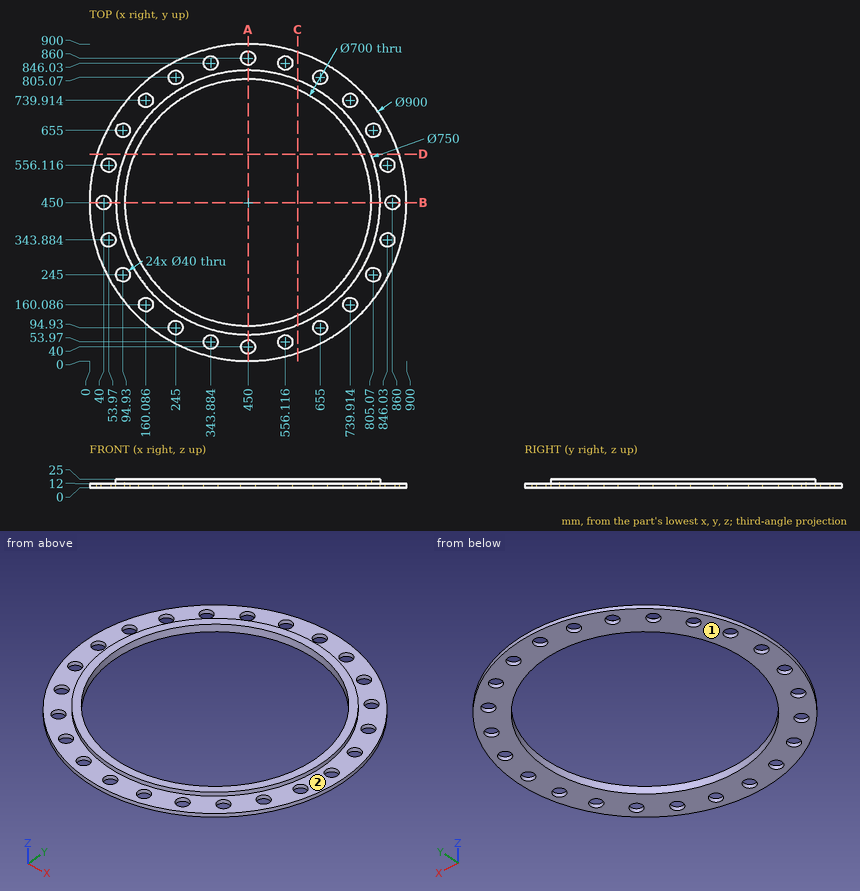
For this review, use the dimensioned drawing (mm, ordinates from the lowest corner) and the shaded views. A direction names the side the tool comes from. Coordinates: 2 decimals unless noted, no trailing zeros. Loops run counter-clockwise (first coordinate to the right, second up) from the corner with the lowest first, then second, coordinate; pieces in that order, holes last. Notation, with made-up numbers: (60, 67.5) -> (105, 67.5) arc R18 cw to (105, 101.5) -> close; hole circle Ø11 at (89, 46). An arc over 180 degrees is marked (long way). Use a Markdown table: item, result. Add a question column.
1. To check wall thickness, follow line 1 (X direction, y = 847, z = 7.25) (1 decimal); line 2 (X direction, y = 860, z = 3) (1 decimal); line 3 (Z direction, x = 248.5, y = 848). State the ranges of each line that lie inside material, in increasing order.
2. Add section A-A on x = 450. Write out the cut boundary in (y, z), plus the area to 3 significant figures.
3. Clearance check with flat-ended pins moving along their axes: pin 1 Ø10 at (y, z) = (162, 11.5) entering from -X; pin 2 Ø24 at (x, y) = (94.93, 245) entering from +Z; pin 3 Ø2 at (x, z) = (487.5, 3.5) entering from -Y; pin 4 Ø1 at (y, z) = (552.5, 6.5) entering from +X. State where each tip first meets the part, or that it passes through.
4. Machinability: for the marked faces 1 and 2, which of the approach directions +Z, -Z, +X, -X, +Y, -Y give a long, thin tool a straight path to every point of the face, cutting with its end or side? Answer none if there is none.
5. Add section C-C on x = 591. Write out the cut boundary in (y, z).
6. Add section D-D on y = 587.5. Write out the cut boundary in (x, z), plus the area to 3 significant figures.
Returned:
| question | item | result |
|---|---|---|
| 1 | line 1 | x = 238.1 to 323.9, 363.9 to 434.8, 465.2 to 536.1, 576.1 to 661.9 |
| 1 | line 2 | x = 264.5 to 329.6, 358.2 to 430, 470 to 541.8, 570.4 to 635.5 |
| 1 | line 3 | z = 0 to 12 |
| 2 | outline | (0, 0) -> (20, 0) -> (20, 12) -> (0, 12) -> close; (60, 0) -> (100, 0) -> (100, 25) -> (75, 25) -> (75, 12) -> (60, 12) -> close; (800, 0) -> (840, 0) -> (840, 12) -> (825, 12) -> (825, 25) -> (800, 25) -> close; (880, 0) -> (900, 0) -> (900, 12) -> (880, 12) -> close |
| 2 | area | 2,090 mm² |
| 3 | pin 1 | stops at x = 100.13 |
| 3 | pin 2 | passes through |
| 3 | pin 3 | stops at y = 1.48 |
| 3 | pin 4 | stops at x = 888.29 |
| 4 | face 1 | -Z, +X, -X, +Y, -Y |
| 4 | face 2 | +Z |
| 5 | outline | (22.66, 0) -> (129.66, 0) -> (129.66, 25) -> (102.52, 25) -> (102.52, 12) -> (22.66, 12) -> close; (770.34, 0) -> (877.34, 0) -> (877.34, 12) -> (797.48, 12) -> (797.48, 25) -> (770.34, 25) -> close |
| 6 | outline | (21.52, 0) -> (128.14, 0) -> (128.14, 25) -> (101.12, 25) -> (101.12, 12) -> (21.52, 12) -> close; (771.86, 0) -> (878.48, 0) -> (878.48, 12) -> (798.88, 12) -> (798.88, 25) -> (771.86, 25) -> close |
| 6 | area | 3,260 mm² |
